Here's how the part is built. I have some questions about the finished solid (model axes, mm). Round coordinates to 2 decimals unless told otherwise and drop trailing zeros. Loops run counter-clockwise (first coordinate to the right, second up) from the corner with the lowest first, then second, coordinate; pieces in that order, holes last. Notation, with made-up numbers: M -0.5,58 L 25.5,58 A27 cw 25.5,78 Z; hole C 3.5,-4.5 d10. An arc over 180 degrees is marked long. Use a Markdown table: item, result.
```python
from build123d import *

# Parameters (mm, degrees)
SKETCH_1_W      = 60
SKETCH_1_H      = 15
EXTRUDE_1_DEPTH = 3


with BuildPart() as part:
    # 草图1 → 凸台-拉伸1 (new body)
    with BuildSketch(Plane.XY):
        Rectangle(SKETCH_1_W, SKETCH_1_H)
    extrude(amount=EXTRUDE_1_DEPTH)

    # 草图2 → M3 十字切槽平头螺钉锥孔1 (revolve, cut)
    with BuildSketch(Plane(origin=(-14.533919383, 0.114773803, 0), x_dir=(0, 1, 0), z_dir=(1, 0, 0))):
        Polygon((0, 0), (0, 3), (1.7, 3), (1.7, 1.45), (3.15, 0), align=None)
    revolve(axis=Axis((-14.533919383, 0.114773803, -6.35), (0, 0, 1)), mode=Mode.SUBTRACT)


solid = part.part
```
Q1. Will these pins go through, and if not, where does the flat tip stop? P1, Ø2, axis at x = -14.53, y = 0.11, coming from the -Z side; P2, Ø3, axis at x = 13.5, y = 3.5, coming from the -Z side.
Return value:
| item | result |
|---|---|
| P1 | passes through |
| P2 | stops at z = 0 |
Q2. Imagine slicing it at A-A, the plane z = 0.85. Please give me the cut outline in (x, y), then the cut area to 3 significant figures.
Return value:
| item | result |
|---|---|
| outline | M -30,-7.5 L 30,-7.5 L 30,7.5 L -30,7.5 Z; hole C -14.53,0.11 d4.6 |
| area | 883 mm^2 |
Q3. I need wall thicknesses on line 1 (Y direction, x = -15, z = 1). Which ranges of the line are inside material? Lowest first, please. Write a range as from..to.
Return value:
| item | result |
|---|---|
| line 1 | y = -7.5..-1.98, 2.21..7.5 |
Q4. We'd pull the mould along X, two halves only. Please class faces 1 (the cylindrical face through (-16.22, -0.11, 2.21)), 2 (the flat face through (0, 7.5, 1)), 3 (the flat face through (30, 0, 1)): pulls with the +X half, pulls with the -X half, needs draft (parallel to the pull), parting line crosses it, or undercut.
Return value:
| item | result |
|---|---|
| face 1 | undercut |
| face 2 | needs draft |
| face 3 | pulls with the +X half |
